Here's how the part is built. I have some questions about the finished solid (model axes, mm). Face numbers are marked on the shaded views. Coordinates: 2 decimals unless noted, no trailing zeros. Loops run counter-clockwise (first coordinate to the right, second up) from the corner with the lowest first, then second, coordinate; pieces in that order, holes last. Notation, with made-up numbers: (48.5, 48) - (78.5, 48) arc R25 cw to (78.5, 77) - close; hole circle Ø11 at (27, 33.5). An arc over 180 degrees is marked (long way). Use a Markdown table: item, result.
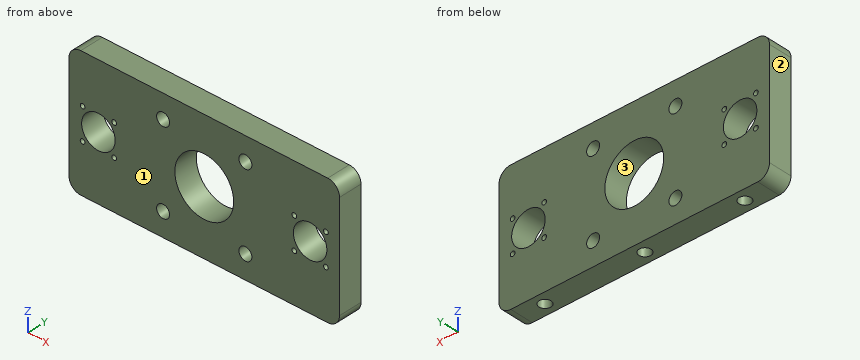
```python
from build123d import *

# Parameters (mm, degrees)
SKETCH1_W              = 230
SKETCH1_H              = 110
BOSS_EXTRUDE1_DEPTH    = 20
SKETCH2_R              = 14.25
CUT_EXTRUDE2_DEPTH     = 256.734237051
SKETCH3_R              = 2
CUT_EXTRUDE3_DEPTH     = 256.734237051
LPATTERN1_COUNT        = 2
LPATTERN1_PITCH        = 180
FILLET1_R              = 10
SKETCH4_R              = 25
SKETCH4_R_2            = 5.5
CUT_EXTRUDE4_DEPTH     = 100
M12_TAPPED_HOLE2_D     = 10.2
M12_TAPPED_HOLE2_DEPTH = 20
M12_TAPPED_HOLE2_TIP   = 3.064389157


with BuildPart() as part:
    # Sketch1 → Boss-Extrude1 (new body)
    with BuildSketch(Plane(origin=(0, 0, 0), x_dir=(1, 0, 0), z_dir=(0, 1, 0))):
        with Locations((115, 55)):
            Rectangle(SKETCH1_W, SKETCH1_H)
    extrude(amount=BOSS_EXTRUDE1_DEPTH)

    # Sketch2 → Cut-Extrude2 (cut, through all)
    with BuildSketch(Plane(origin=(0, 20, 0), x_dir=(1, 0, 0), z_dir=(0, 1, 0))):
        with Locations(Location((25, 55, 0), (0, 0, 270))):
            Circle(SKETCH2_R)
        with Locations(Location((205, 55, 0), (0, 0, 270))):
            Circle(SKETCH2_R)
    extrude(amount=-CUT_EXTRUDE2_DEPTH, mode=Mode.SUBTRACT)

    # Sketch3 → Cut-Extrude3 (cut, through all)
    with BuildSketch(Plane(origin=(0, 20, 0), x_dir=(1, 0, 0), z_dir=(0, 1, 0))):
        with Locations(Location((11.564971157, 68.435028843, 0), (0, 0, 270))):
            Circle(SKETCH3_R)
        with Locations(Location((38.435028843, 68.435028843, 0), (0, 0, 270))):
            Circle(SKETCH3_R)
        with Locations(Location((38.435028843, 41.564971157, 0), (0, 0, 270))):
            Circle(SKETCH3_R)
        with Locations(Location((11.564971157, 41.564971157, 0), (0, 0, 270))):
            Circle(SKETCH3_R)
    cut_extrude3 = extrude(amount=-CUT_EXTRUDE3_DEPTH, mode=Mode.SUBTRACT)

    # LPattern1: Cut-Extrude3 ×2
    with Locations(*[(i * LPATTERN1_PITCH, 0, 0) for i in range(1, LPATTERN1_COUNT)]):
        add(cut_extrude3, mode=Mode.SUBTRACT)

    # Fillet1
    fillet1_edges = [part.edges().sort_by_distance(p)[0] for p in [
        (0, 10, 0),
        (0, 10, -110),
        (230, 10, -110),
        (230, 10, 0),
    ]]
    fillet(fillet1_edges, radius=FILLET1_R)

    # Sketch4 → Cut-Extrude4 (cut)
    with BuildSketch(Plane(origin=(0, 20, 0), x_dir=(1, 0, 0), z_dir=(0, 1, 0))):
        with Locations(Location((115, 55, 0), (0, 0, 270))):
            Circle(SKETCH4_R)
        with Locations(Location((150, 90, 0), (0, 0, 270))):
            Circle(SKETCH4_R_2)
        with Locations(Location((150, 20, 0), (0, 0, 270))):
            Circle(SKETCH4_R_2)
        with Locations(Location((80, 20, 0), (0, 0, 270))):
            Circle(SKETCH4_R_2)
        with Locations(Location((80, 90, 0), (0, 0, 270))):
            Circle(SKETCH4_R_2)
    extrude(amount=-CUT_EXTRUDE4_DEPTH, mode=Mode.SUBTRACT)

    # M12 Tapped Hole2
    with Locations(Plane(origin=(0, 0, -110), x_dir=(-1, 0, 0), z_dir=(0, 0, -1))):
        with Locations((-200, 10), (-115, 10), (-30, 10)):
            Hole(M12_TAPPED_HOLE2_D / 2, depth=M12_TAPPED_HOLE2_DEPTH)
            with Locations((0, 0, -(M12_TAPPED_HOLE2_DEPTH + M12_TAPPED_HOLE2_TIP / 2))):  # 118° drill point
                Cone(0, M12_TAPPED_HOLE2_D / 2, M12_TAPPED_HOLE2_TIP, mode=Mode.SUBTRACT)


solid = part.part
```
Q1. I want a section at C-C, the plane x = 124.5. Write out the boundary of the cut face in (y, z).
Check values:
| item | result |
|---|---|
| outline | (0, -110) - (20, -110) - (20, -78.12) - (0, -78.12) - close; (0, -31.88) - (20, -31.88) - (20, 0) - (0, 0) - close |
Q2. I want a section at D-D, the plane x = 93. Write out the boundary of the cut face in (y, z), then the cut area to 3 significant figures.
Check values:
| item | result |
|---|---|
| outline | (0, -110) - (20, -110) - (20, -66.87) - (0, -66.87) - close; (0, -43.13) - (20, -43.13) - (20, 0) - (0, 0) - close |
| area | 1,730 mm^2 |
Q3. I want a section at A-A, the plane z = -20. Write out the boundary of the cut face in (x, y), then the cut area to 3 significant figures.
Check values:
| item | result |
|---|---|
| outline | (0, 0) - (74.5, 0) - (74.5, 20) - (0, 20) - close; (85.5, 0) - (144.5, 0) - (144.5, 20) - (85.5, 20) - close; (155.5, 0) - (230, 0) - (230, 20) - (155.5, 20) - close |
| area | 4,160 mm^2 |
Q4. If we mould it in two halves opening along X, with no side actions, what happens to the marked faces 1, 2 and 3? For each: pulls with the +X half, pulls with the -X half, needs draft (parallel to the pull), parting line crosses it, or undercut.
Check values:
| item | result |
|---|---|
| face 1 | needs draft |
| face 2 | pulls with the -X half |
| face 3 | undercut |
Q5. Will these pins go through, and if not, where does the flat tip stop? P1, Ø14.5, axis at x = 80, z = -90, coming from the +Y side; P2, Ø3, axis at x = 38.44, z = -68.44, coming from the -Y side.
Check values:
| item | result |
|---|---|
| P1 | y = 20 |
| P2 | through |
Q6. Please list where these lines run through material, in increasing order: L1, parallel to X at y = 7.25, z = -55; L2, parallel to X at y = 15.75, z = -90; L3, parallel to Y at x = 200, z = -93.75. Write a range as from..to.
Check values:
| item | result |
|---|---|
| L1 | 0..10.75, 39.25..90, 140..190.75, 219.25..230 |
| L2 | 0..74.5, 85.5..144.5, 155.5..230 |
| L3 | 0..4.9, 15.1..20 |
Q7. I want a section at B-B, the plane z = -55. Write out the boundary of the cut face in (x, y).
Check values:
| item | result |
|---|---|
| outline | (0, 0) - (10.75, 0) - (10.75, 20) - (0, 20) - close; (39.25, 0) - (90, 0) - (90, 20) - (39.25, 20) - close; (140, 0) - (190.75, 0) - (190.75, 20) - (140, 20) - close; (219.25, 0) - (230, 0) - (230, 20) - (219.25, 20) - close |
